The figure shows three views and two pictorial views of one solid part (mm, origin at its lowest corner). Answer the questions. Round coordinates to 2 decimals unless told otherwise and drop trailing zeros. Write each loop counter-clockwise with the first axis right and the second up, starting at its lowest first coordinate (ties: lowest second). Pieces come first, ordered by that corner, then holes. Notation, with made-up numbers: M -39.75,36.25 L 10.25,36.25 A27 cw 10.25,71.25 Z; hole C 34.25,71.5 d6. An arc over 180 degrees is marked long. One line per item, written item: value. Start each with the question number.
Q1. Consider probe 1 along Y at (x, z) = (4, 0.8); probe 2 along Y at (x, z) = (5.25, 1.9) (1 decimal); probe 3 along X at (y, z) = (3.75, 2.9) (1 decimal). Determine where each line is inside the solid, lowest interval first.
Q2. Find section D-D (x = 7.25). Write down the section's boundary in (y, z).
Q3. Find section C-C (x = 3.25). Write down the section's boundary in (y, z).
Q4. Find section B-B (y = 3). Write down the section's boundary in (x, z) (1 decimal).
Q5. The mould has two halves that part along Y. Classify the marked faces 1, 2 and 3: released by +Y, released by -Y, zero draft, split by the parting line, or undercut.
Q6. Find section A-A (z = 2.1). Write down the section's boundary in (x, y), and give its area (3 significant figures).
Q7. Given pin 1 Ø1.5 at (x, z) = (7, 2) entering from -Y (1 decimal); pin 2 Ø1.5 at (x, z) = (6.5, 1.5) entering from +Y, each flat-ended and moving along its own axis, determine where each tip first touches the part or whether it passes through.
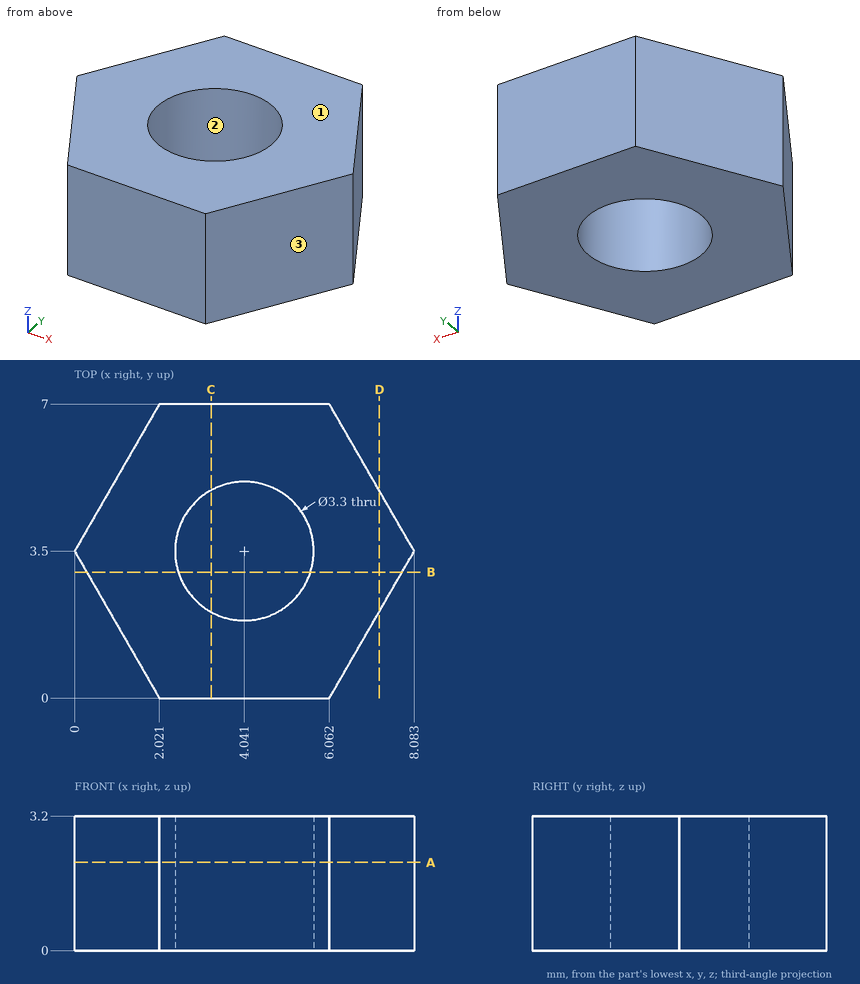
The answers:
1. probe 1: 0 to 1.85, 5.15 to 7
1. probe 2: 0 to 2.4, 4.6 to 7
1. probe 3: 0.1 to 2.4, 5.7 to 7.9
2. outline: M 2.06,0 L 4.94,0 L 4.94,3.2 L 2.06,3.2 Z
3. outline: M 0,0 L 2.05,0 L 2.05,3.2 L 0,3.2 Z; M 4.95,0 L 7,0 L 7,3.2 L 4.95,3.2 Z
4. outline: M 0.3,0 L 2.5,0 L 2.5,3.2 L 0.3,3.2 Z; M 5.6,0 L 7.8,0 L 7.8,3.2 L 5.6,3.2 Z
5. face 1: zero draft
5. face 2: undercut
5. face 3: released by -Y
6. outline: M 0,3.5 L 2.02,0 L 6.06,0 L 8.08,3.5 L 6.06,7 L 2.02,7 Z; hole C 4.04,3.5 d3.3
6. area: 33.9 mm2
7. pin 1: y = 0.3
7. pin 2: y = 7
